```python
from build123d import *

# Parameters (mm, degrees)
EXTRUDE_THIN1_DEPTH = 500
SKETCH3_W           = 455
SKETCH3_H           = 40
EXTRUDE1_DEPTH      = 1
SKETCH7_W           = 455
SKETCH7_H           = 40
EXTRUDE3_DEPTH      = 1
SKETCH8_W           = 43
SKETCH8_H           = 1
CUT_EXTRUDE1_DEPTH  = 20
SKETCH9_R           = 2.75
CUT_EXTRUDE2_DEPTH  = 10


with BuildPart() as part:
    # Sketch2 → Extrude-Thin1 (new, symmetric)
    with BuildSketch(Plane(origin=(0, 0, 0), x_dir=(0, 0, -1), z_dir=(1, 0, 0))):
        Polygon((-22, -50), (-22, -40), (0, -40), (0, 0), (-455, 0), (-455, -40), (-454, -40), (-454, -1), (-1, -1), (-1, -39), (-23, -39), (-23, -50), align=None)
    extrude(amount=EXTRUDE_THIN1_DEPTH, both=True)

    # Sketch3 → Extrude1 (add)
    with BuildSketch(Plane(origin=(500, 0, 0), x_dir=(0, 0, -1), z_dir=(1, 0, 0))):
        with Locations((-227.5, -20)):
            Rectangle(SKETCH3_W, SKETCH3_H)
    extrude(amount=EXTRUDE1_DEPTH)

    # Sketch7 → Extrude3 (add)
    with BuildSketch(Plane.ZY.offset(500)):
        with Locations((227.5, -20)):
            Rectangle(SKETCH7_W, SKETCH7_H)
    extrude(amount=EXTRUDE3_DEPTH)

    # Sketch8 → Cut-Extrude1 (cut)
    with BuildSketch(Plane.XZ.offset(50)):
        with Locations((478.5, 22.5)):
            Rectangle(SKETCH8_W, SKETCH8_H)
        with Locations((-478.5, 22.5)):
            Rectangle(SKETCH8_W, SKETCH8_H)
    extrude(amount=-CUT_EXTRUDE1_DEPTH, mode=Mode.SUBTRACT)

    # Sketch9 → Cut-Extrude2 (cut)
    with BuildSketch(Plane.XZ.offset(40)):
        with Locations(Location((491, 15, 0), (0, 0, 270))):
            Circle(SKETCH9_R)
        with Locations(Location((-491, 15, 0), (0, 0, 270))):
            Circle(SKETCH9_R)
    extrude(amount=-CUT_EXTRUDE2_DEPTH, mode=Mode.SUBTRACT)


solid = part.part
```
Check sheet for the modelled part. Datum: model origin and axes. Units: mm. A direction names the side the tool comes from. Coordinates: 2 decimals unless noted, no trailing zeros. Loops run counter-clockwise (first coordinate to the right, second up) from the corner with the lowest first, then second, coordinate; pieces in that order, holes last.
1) Sectioned sample at A-A (y = -19). Record the boundary of the cut face in (x, z), and give its area (3 significant figures).
2) Gauge pin test, flat ends, axial feed: pin 1 (10 mm diameter, centred on x = -347, z = 340.5, fed in from -Y); pin 2 (5.5 mm diameter, centred on x = 60, y = -44.5, fed in from +Z); pin 3 (3 mm diameter, centred on x = 26.5, y = -47, fed in from -Z). Record the tip position at first contact, or that the pin passes through.
3) Sectioned sample at B-B (z = 339.5). Record the boundary of the cut face in (x, y).
4) Material ranges on probe 1 along X at (y, z) = (-39.5, 15); probe 2 along Z at (x, y) = (491, -39.4); probe 3 along Z at (x, y) = (-36, -36), recorded low to high.
5) Access from +Z, -Z, +X, -X, +Y, -Y to the whole of each face (thin tool, end or side, straight path). Record for faces 1 (the face through (7, -20, 1)), 2 (the face through (7, -21, 454)), 3 (the face through (501, -20, 231)).
6) Release check for a two-part mould opening along Z. For faces 4 (the face through (7, -20, 455)), 5 (the face through (7, -1, 231)), 6 (the face through (7, -20, 0)), 7 (the face through (7, 0, 224)) record: released by +Z, released by -Z, zero draft, split by the parting line, or undercut.
7) Sectioned sample at C-C (x = -121.5). Record the boundary of the cut face in (y, z), and give its area (3 significant figures).
Check sheet entries:
1. outline: (-501, 0) - (501, 0) - (501, 455) - (-501, 455) - close; hole (-500, 1) - (500, 1) - (500, 454) - (-500, 454) - close
1. area: 2,910 mm2
2. pin 1: stops at y = -1
2. pin 2: stops at z = 23
2. pin 3: stops at z = 22
3. outline: (-501, -40) - (-500, -40) - (-500, -1) - (500, -1) - (500, -40) - (501, -40) - (501, 0) - (-501, 0) - close
4. probe 1: x = -501 to -493.75, -488.25 to 488.25, 493.75 to 501
4. probe 2: z = 0 to 12.25, 17.75 to 22, 454 to 455
4. probe 3: z = 0 to 1, 454 to 455
5. face 1: none
5. face 2: -Y
5. face 3: +Z, -Z, +X, +Y, -Y
6. face 4: released by +Z
6. face 5: undercut
6. face 6: released by -Z
6. face 7: zero draft
7. outline: (-50, 22) - (-40, 22) - (-40, 0) - (0, 0) - (0, 455) - (-40, 455) - (-40, 454) - (-1, 454) - (-1, 1) - (-39, 1) - (-39, 23) - (-50, 23) - close
7. area: 565 mm2
